Model file for the job. Use its own axes, mm. Face numbers are marked on the shaded views. A direction names the side the tool comes from. Round coordinates to 2 decimals unless told otherwise and drop trailing zeros. Order: outer loops, then holes, each group sorted by start corner. A loop starts at its lowest first (then second) coordinate and runs counter-clockwise, first axis right, second up. Notation, with made-up numbers: (64.25, 36.25) - (112.25, 36.25) arc R18 cw to (112.25, 54.25) - close; hole circle Ø5 at (54.5, 38.25). An arc over 180 degrees is marked (long way). Write item = value, one per line. Start each with the question number.
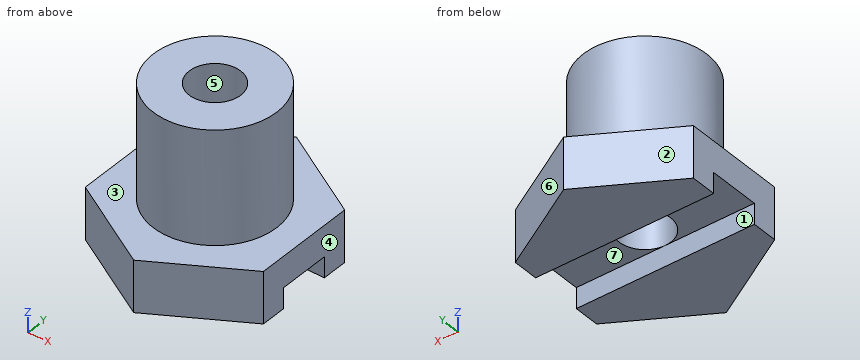
from build123d import *

# Parameters (mm, degrees)
HEX_FLANGE_DEPTH          = 5
BOSS_SKETCH_12_R          = 6
CYLINDRICAL_BOSS_12_DEPTH = 11
FLANGE_SLOT_SKETCH_W      = 17.320508076
FLANGE_SLOT_SKETCH_H      = 5
FLANGE_SLOT_CUT_DEPTH     = 2
BORE_SKETCH_5_R           = 2.5
BORE_5_DEPTH              = 20.261360284


with BuildPart() as part:
    # Hex Flange Sketch → Hex Flange (new body)
    with BuildSketch(Plane.XY):
        Polygon((0, 10), (-8.660254038, 5), (-8.660254038, -5), (0, -10), (8.660254038, -5), (8.660254038, 5), align=None)
    extrude(amount=HEX_FLANGE_DEPTH)

    # Boss Sketch Ø12 → Cylindrical Boss Ø12 (add)
    with BuildSketch(Plane.XY.offset(5)):
        Circle(BOSS_SKETCH_12_R)
    extrude(amount=CYLINDRICAL_BOSS_12_DEPTH)

    # Flange Slot Sketch → Flange Slot Cut (cut)
    with BuildSketch(Plane(origin=(0, 0, 0), x_dir=(-1, 0, 0), z_dir=(0, 0, -1))):
        Rectangle(FLANGE_SLOT_SKETCH_W, FLANGE_SLOT_SKETCH_H)
    extrude(amount=-FLANGE_SLOT_CUT_DEPTH, mode=Mode.SUBTRACT)

    # Bore Sketch Ø5 → Bore Ø5 (cut, through all)
    with BuildSketch(Plane(origin=(0, 0, 2), x_dir=(-1, 0, 0), z_dir=(0, 0, -1))):
        Circle(BORE_SKETCH_5_R)
    extrude(amount=-BORE_5_DEPTH, mode=Mode.SUBTRACT)


solid = part.part
Item 1: Drop flat-ended pins along their axis: pin 1 (1.5 mm diameter, centred on x = 4, y = 0.5, fed in from -Z); pin 2 (4 mm diameter, centred on x = 4, z = 8, fed in from -Y); pin 3 (1.5 mm diameter, centred on y = 3, z = 7, fed in from -X). Give the stop position or say it passes through.
Item 2: Saw through at D-D, the plane y = -3.75. Give the cut face in (x, z).
Item 3: Saw through at C-C, the plane x = 3. Give the cut face in (y, z), then the cut area to 3 significant figures.
Item 4: Probe L1, parallel to Y at x = 0, z = 5.75; L2, parallel to Y at x = 0.5, z = 9.75; L3, parallel to Z at x = 1.75, y = 8.5. List the from-to ranges inside material, lowest first.
Item 5: Which spindle directions (+Z, -Z, +X, -X, +Y, -Y) get a long thin tool onto all of the face, cutting with end or side? Do the marked faces 1, 2 and 3. Say none if no direction does.
Item 6: Saw through at A-A, the plane y = 0. Give the cut face in (x, z).
Item 7: Mould opens along Y. For the marked faces 4, 5, 6 and 7 say: +Y half, -Y half, draft (parallel to the pull), parting line (faces both ways), or undercut.
Item 8: Saw through at B-B, the plane z = 3. Give the cut face in (x, y).
Check sheet entries:
q1.pin_1 = 2
q1.pin_2 = -5.66
q1.pin_3 = -5.56
q2.outline = (-8.66, 0) - (8.66, 0) - (8.66, 5) - (4.68, 5) - (4.68, 16) - (-4.68, 16) - (-4.68, 5) - (-8.66, 5) - close
q3.outline = (-8.27, 0) - (-2.5, 0) - (-2.5, 2) - (2.5, 2) - (2.5, 0) - (8.27, 0) - (8.27, 5) - (5.2, 5) - (5.2, 16) - (-5.2, 16) - (-5.2, 5) - (-8.27, 5) - close
q3.area = 187 mm2
q4.L1 = -6 to -2.5, 2.5 to 6
q4.L2 = -5.98 to -2.45, 2.45 to 5.98
q4.L3 = 0 to 5
q5.face_1 = -Z, +X, -X
q5.face_2 = +Z, -Z, -X, +Y
q5.face_3 = +Z
q6.outline = (-8.66, 2) - (-2.5, 2) - (-2.5, 16) - (-6, 16) - (-6, 5) - (-8.66, 5) - close; (2.5, 2) - (8.66, 2) - (8.66, 5) - (6, 5) - (6, 16) - (2.5, 16) - close
q7.face_4 = draft
q7.face_5 = undercut
q7.face_6 = +Y half
q7.face_7 = undercut
q8.outline = (-8.66, -5) - (0, -10) - (8.66, -5) - (8.66, 5) - (0, 10) - (-8.66, 5) - close; hole circle Ø5 at (0, 0)
